Work out the finished part from the listing and answer in its coordinate system (mm). Face numbers are marked on the shaded views. Round coordinates to 2 decimals unless told otherwise and drop trailing zeros. Loops run counter-clockwise (first coordinate to the right, second up) from the corner with the lowest first, then second, coordinate; pieces in that order, holes last. Notation, with made-up numbers: (-39.5, 2) - (-19.5, 2) arc R24 cw to (-19.5, 20) - close; hole circle Ø10 at (76, 27.5). An arc over 180 degrees is marked (long way). Answer as CSV lines item,"result". Start each with the question number.
Q1. Section A-A on y = 25 is taken. Write down the section's boundary in (x, z).
Q2. Section D-D on z = 20.5 is taken. Write down the section's boundary in (x, y), then the cut area to 3 significant figures.
Q3. Section B-B on y = 0 is taken. Write down the section's boundary in (x, z), then the cut area to 3 significant figures.
Q4. This flat-tipped pin is pushed along its axis until it touches: pin 1 Ø3 at (x, y) = (-13, 13.5) entering from -Z. Where does it stop, or does it pass through?
Q5. Section C-C on x = 0 is taken. Write down the section's boundary in (y, z), then the cut area to 3 significant figures.
Q6. The mould has two halves that part along X. Classify the marked faces 1, 2 and 3: +X half, -X half, draft (parallel to the pull), parting line (faces both ways), or undercut.
Q7. Straight lines are drawn through the part: L1, parallel to Y at x = 0, z = 11.5; L2, parallel to Z at x = -16, y = 0; L3, parallel to Y at x = -10, z = 2.5. For each, find the intervals that lie inside material, in ascending order. Write a range as [from, to].
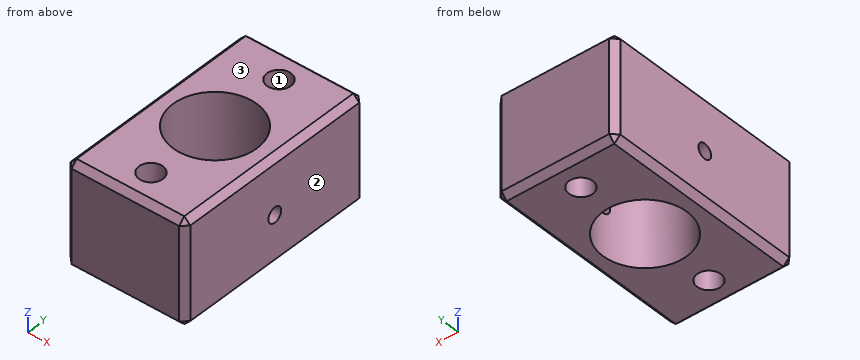
```python
from build123d import *

# Parameters (mm, degrees)
SKETCH_1_W              = 40
SKETCH_1_H              = 70
EXTRUDE_1_DEPTH         = 35
SKETCH_2_R              = 14
CUT_EXTRUDE_1_DEPTH     = 64
SKETCH_4_R              = 4
CUT_EXTRUDE_3_DEPTH     = 59
HOLE_WIZARD_M6_1_REACH  = 58.279
HOLE_WIZARD_M6_1_BORE_R = 2.5
CHAMFER_1_SIZE          = 2


with BuildPart() as part:
    # 草图1 → 凸台-拉伸1 (new body)
    with BuildSketch(Plane.XY):
        Rectangle(SKETCH_1_W, SKETCH_1_H)
    extrude(amount=EXTRUDE_1_DEPTH)

    # 草图2 → 切除-拉伸1 (cut)
    with BuildSketch(Plane.XY.offset(35)):
        Circle(SKETCH_2_R)
    extrude(amount=-CUT_EXTRUDE_1_DEPTH, mode=Mode.SUBTRACT)

    # 草图4 → 切除-拉伸3 (cut)
    with BuildSketch(Plane.XY.offset(35)):
        with Locations((0, 25)):
            Circle(SKETCH_4_R)
    cut_extrude_3 = extrude(amount=-CUT_EXTRUDE_3_DEPTH, mode=Mode.SUBTRACT)

    # M6 螺纹孔1 bore (on position points) → M6 螺纹孔1 (cut, up to next)
    with BuildSketch(Plane(origin=(-20, 0, 16.498820141), x_dir=(0, 0, -1), z_dir=(-1, 0, 0)), mode=Mode.PRIVATE) as hole_wizard_m6_1_sk1:
        Circle(HOLE_WIZARD_M6_1_BORE_R)
    hole_wizard_m6_1_tool1 = extrude(hole_wizard_m6_1_sk1.sketch, amount=-HOLE_WIZARD_M6_1_REACH, mode=Mode.PRIVATE) & part.part
    hole_wizard_m6_1 = hole_wizard_m6_1_tool1.solids().sort_by_distance((-20, 0, 16.49882))[0]
    add(hole_wizard_m6_1, mode=Mode.SUBTRACT)

    # 镜向2: 切除-拉伸3 across plane
    add(cut_extrude_3.mirror(Plane.ZX), mode=Mode.SUBTRACT)

    # 镜向3: M6 螺纹孔1 across plane
    add(hole_wizard_m6_1.mirror(Plane(origin=(0, 0, 0), x_dir=(0, 0, 1), z_dir=(1, 0, 0))), mode=Mode.SUBTRACT)

    # 倒角1
    chamfer_1_edges = [part.edges().sort_by_distance(p)[0] for p in [
        (-20, 0, 35),
        (0, -35, 35),
        (20, 0, 35),
        (0, -35, 0),
        (-20, 0, 0),
        (0, 35, 0),
        (20, 0, 0),
        (20, -35, 17.5),
        (-20, -35, 17.5),
        (-20, 35, 17.5),
        (20, 35, 17.5),
        (0, 35, 35),
    ]]
    chamfer(chamfer_1_edges, length=CHAMFER_1_SIZE)


solid = part.part
```
Findings:
1,outline,"(-20, 2) - (-18, 0) - (-4, 0) - (-4, 35) - (-18, 35) - (-20, 33) - close; (4, 0) - (18, 0) - (20, 2) - (20, 33) - (18, 35) - (4, 35) - close"
2,outline,"(-20, -33) - (-18, -35) - (18, -35) - (20, -33) - (20, 33) - (18, 35) - (-18, 35) - (-20, 33) - close; hole circle Ø28 at (0, 0); hole circle Ø8 at (0, -25); hole circle Ø8 at (0, 25)"
2,area,"2,080 mm^2"
3,outline,"(-20, 2) - (-18, 0) - (-14, 0) - (-14, 14) - (-20, 14) - close; (-20, 19) - (-14, 19) - (-14, 35) - (-18, 35) - (-20, 33) - close; (14, 0) - (18, 0) - (20, 2) - (20, 14) - (14, 14) - close; (14, 19) - (20, 19) - (20, 33) - (18, 35) - (14, 35) - close"
3,area,"352 mm^2"
4,pin 1,"stops at z = 0"
5,outline,"(-35, 2) - (-33, 0) - (-29, 0) - (-29, 35) - (-33, 35) - (-35, 33) - close; (-21, 0) - (-14, 0) - (-14, 35) - (-21, 35) - close; (14, 0) - (21, 0) - (21, 35) - (14, 35) - close; (29, 0) - (33, 0) - (35, 2) - (35, 33) - (33, 35) - (29, 35) - close"
5,area,"902 mm^2"
6,face 1,"undercut"
6,face 2,"+X half"
6,face 3,"draft"
7,L1,"y = [-35, -29], [-21, -14], [14, 21], [29, 35]"
7,L2,"z = [0, 14], [19, 35]"
7,L3,"y = [-35, -9.8], [9.8, 35]"
